For this review, take the finished solid that the model builds, in its own axes (mm). Face numbers are marked on the shaded views. A direction names the side the tool comes from. Round coordinates to 2 decimals unless told otherwise and drop trailing zeros. Order: outer loops, then holes, each group sorted by start corner. A loop starts at its lowest first (then second) coordinate and runs counter-clockwise, first axis right, second up. Notation, with made-up numbers: (-30, -35.5) - (-18, -35.5) arc R16 cw to (-18, -4.5) - close; hole circle Ø7 at (64, -1.75). An arc over 180 degrees is marked (long way). Write each question's results on one line, items separated by ' | '. Start each with the question number.
(1) Insertion check: pin 1 Ø2 at (y, z) = (0.5, 4.5) entering from +X; pin 2 Ø4 at (y, z) = (-4, 14) entering from -X; pin 3 Ø2 at (x, y) = (3.5, 4) entering from +Z. Each pin has a flat end and moves straight along its axis. Give the tip position at first contact, or say it passes through.
(2) For the marked faces 1 and 2, list the 3-axis set-ups (+Z, -Z, +X, -X, +Y, -Y) from which the entire face can be reached by the end or side of a thin tool; tool diameter is ignored.
(3) Take a section at C-C, the plane y = 0. Give the boundary of the cut face in (x, z), plus the area to 3 significant figures.
(4) For L1, parallel to Z at x = -3.25, y = -4.25; L2, parallel to Z at x = 0.75, y = 0.25; L3, parallel to Y at x = 0, z = 3.25, list the stretches that pass through material, from the lowest coordinate up. Write a range as from..to.
(5) Take a section at A-A, the plane x = 0. Give the boundary of the cut face in (y, z), plus the area to 3 significant figures.
(6) Draft analysis for pull direction Y (two halves, no side actions). For the marked faces 3, 4, 5 and 6, state which applies: pulls with the +Y half, pulls with the -Y half, needs draft (parallel to the pull), parting line crosses it, or undercut.
(7) Take a section at B-B, the plane z = 12.5. Give the boundary of the cut face in (x, y).
```python
from build123d import *

# Parameters (mm, degrees)
SKETCH_1_R          = 6
EXTRUDE_1_DEPTH     = 1.4
SKETCH_2_R          = 3
EXTRUDE_2_DEPTH     = 15
FILLET_1_R          = 0.5
CUT_EXTRUDE_1_DEPTH = 2
CHAMFER_1_SIZE      = 0.5


with BuildPart() as part:
    # 草图1 → 凸台-拉伸1 (new body)
    with BuildSketch(Plane.XY):
        Circle(SKETCH_1_R)
    extrude(amount=EXTRUDE_1_DEPTH)

    # 草图2 → 凸台-拉伸2 (add)
    with BuildSketch(Plane.XY.offset(1.4)):
        Circle(SKETCH_2_R)
    extrude(amount=EXTRUDE_2_DEPTH)

    # 圆角1
    fillet_1_edges = [part.edges().sort_by_distance(p)[0] for p in [
        (-6, 0, 0),
    ]]
    fillet(fillet_1_edges, radius=FILLET_1_R)

    # 草图3 → 切除-拉伸1 (cut)
    with BuildSketch(Plane(origin=(0, 0, 0), x_dir=(-1, 0, 0), z_dir=(0, 0, -1))):
        Polygon((0.749542431, -2.184380799), (2.266500479, -0.443067613), (1.516958048, 1.741313186), (-0.749542431, 2.184380799), (-2.266500479, 0.443067613), (-1.516958048, -1.741313186), align=None)
    extrude(amount=-CUT_EXTRUDE_1_DEPTH, mode=Mode.SUBTRACT)

    # 倒角1
    chamfer_1_edges = [part.edges().sort_by_distance(p)[0] for p in [
        (-3, 0, 16.4),
    ]]
    chamfer(chamfer_1_edges, length=CHAMFER_1_SIZE)


solid = part.part
```
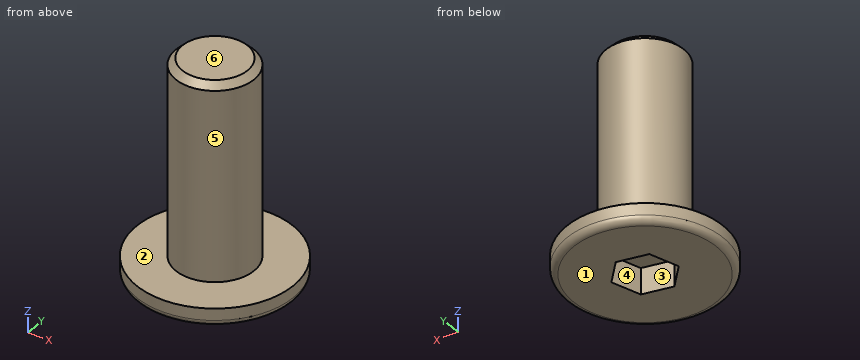
Results below:
1) pin 1: stops at x = 3 | pin 2: stops at x = -2.24 | pin 3: stops at z = 1.4
2) face 1: -Z, +X, -X, +Y, -Y | face 2: +Z
3) outline: (-6, 0.5) arc R0.5 ccw to (-5.5, 0) - (-2.11, 0) - (-2.11, 2) - (2.11, 2) - (2.11, 0) - (5.5, 0) arc R0.5 ccw to (6, 0.5) - (6, 1.4) - (3, 1.4) - (3, 15.9) - (2.5, 16.4) - (-2.5, 16.4) - (-3, 15.9) - (-3, 1.4) - (-6, 1.4) - close | area: 98.0 mm^2
4) L1: z = 0..1.4 | L2: z = 2..16.4 | L3: y = -3..3
5) outline: (-6, 0.5) arc R0.5 ccw to (-5.5, 0) - (-2.04, 0) - (-2.04, 2) - (2.04, 2) - (2.04, 0) - (5.5, 0) arc R0.5 ccw to (6, 0.5) - (6, 1.4) - (3, 1.4) - (3, 15.9) - (2.5, 16.4) - (-2.5, 16.4) - (-3, 15.9) - (-3, 1.4) - (-6, 1.4) - close | area: 98.3 mm^2
6) face 3: undercut | face 4: undercut | face 5: parting line crosses it | face 6: needs draft
7) outline: circle Ø6 at (0, 0)
